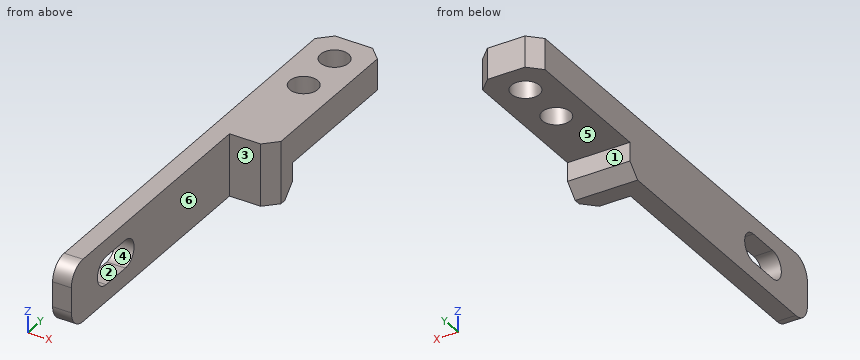
```python
from build123d import *

# Parameters (mm, degrees)
SKETCH1_W            = 10
SKETCH1_H            = 70
BOSS_EXTRUDE1_DEPTH  = 5
SKETCH2_W            = 7
SKETCH2_H            = 41
CUT_EXTRUDE1_DEPTH   = 37.742346142
SKETCH3_W            = 5
SKETCH3_H            = 24
CUT_EXTRUDE2_DEPTH   = 37.742346142
CUT_EXTRUDE3_DEPTH   = 37.742346142
FILLET1_R            = 3
M4_CLEARANCE_HOLE1_D = 4.5
CHAMFER1_SIZE        = 2


with BuildPart() as part:
    # Sketch1 → Boss-Extrude1 (new, symmetric)
    with BuildSketch(Plane.XY):
        Rectangle(SKETCH1_W, SKETCH1_H)
    extrude(amount=BOSS_EXTRUDE1_DEPTH, both=True)

    # Sketch2 → Cut-Extrude1 (cut, through all)
    with BuildSketch(Plane.XY.offset(5)):
        with Locations((1.5, -14.5)):
            Rectangle(SKETCH2_W, SKETCH2_H)
    extrude(amount=-CUT_EXTRUDE1_DEPTH, mode=Mode.SUBTRACT)

    # Sketch3 → Cut-Extrude2 (cut, through all)
    with BuildSketch(Plane(origin=(5, 0, 0), x_dir=(0, 0, -1), z_dir=(1, 0, 0))):
        with Locations((2.5, 23)):
            Rectangle(SKETCH3_W, SKETCH3_H)
    extrude(amount=-CUT_EXTRUDE2_DEPTH, mode=Mode.SUBTRACT)

    # Sketch4 → Cut-Extrude3 (cut, through all)
    with BuildSketch(Plane.ZY.offset(5)):
        with BuildLine():
            Line((2.25, -21), (2.25, -26))
            ThreePointArc((2.25, -26), (0, -28.25), (-2.25, -26))
            Line((-2.25, -26), (-2.25, -21))
            ThreePointArc((-2.25, -21), (0, -18.75), (2.25, -21))
        make_face()
    extrude(amount=-CUT_EXTRUDE3_DEPTH, mode=Mode.SUBTRACT)

    # Fillet1
    fillet1_edges = [part.edges().sort_by_distance(p)[0] for p in [
        (-3.5, -35, 5),
        (-3.5, -35, -5),
    ]]
    fillet(fillet1_edges, radius=FILLET1_R)

    # M4 Clearance Hole1 (through all)
    with Locations(Plane.XY.offset(5)):
        with Locations((0, 30), (0, 22)):
            Hole(M4_CLEARANCE_HOLE1_D / 2)

    # Chamfer1
    chamfer1_edges = [part.edges().sort_by_distance(p)[0] for p in [
        (5, 6, 0),
        (0, 11, -5),
        (-5, 35, 2.5),
        (5, 35, 2.5),
    ]]
    chamfer(chamfer1_edges, length=CHAMFER1_SIZE)


solid = part.part
```
Work out the finished part from the listing and answer in its coordinate system (mm). Face numbers are marked on the shaded views. A direction names the side the tool comes from. Give positions to 0.01 mm unless a question says otherwise; leave off trailing zeros. Write each loop counter-clockwise with the first axis right and the second up, starting at its lowest first coordinate (ties: lowest second). Pieces come first, ordered by that corner, then holes. Notation, with made-up numbers: (-15.5, -14.75) - (16.5, -14.75) arc R27 ccw to (16.5, 13.25) - close; hole circle Ø5 at (66, 9). An arc over 180 degrees is marked (long way). Use one line per item in the form item = value.
1. Each of these flat-tipped pins is pushed along its axis until it touches: pin 1 Ø3 at (x, y) = (3, 13.5) entering from -Z; pin 2 Ø6 at (y, z) = (-17.5, -3) entering from +X; pin 3 Ø5 at (x, y) = (0, 30) entering from +Z; pin 4 Ø1.5 at (x, z) = (0.5, 0) entering from -Y. Where does it stop, or does it pass through?
Filled in:
pin_1 = 0
pin_2 = -2
pin_3 = 5
pin_4 = 6
2. Consider L1, parallel to Y at x = 0, z = 1.3; L2, parallel to Z at x = -2.5, y = -25; L3, parallel to X at y = -1.5, z = 0. Determine where each line is inside the solid, lowest interval first.
Filled in:
L1 = 6 to 19.75, 24.25 to 27.75, 32.25 to 35
L2 = -5 to -2.25, 2.25 to 5
L3 = -5 to -2
3. A cutting plane is placed at D-D (x = 4). Write down the section's boundary in (y, z).
Filled in:
outline = (7, -5) - (9, -5) - (11, -3) - (11, 0) - (34, 0) - (34, 5) - (7, 5) - close
4. A cutting plane is placed at B-B (x = 0). Write down the section's boundary in (y, z).
Filled in:
outline = (6, -5) - (9, -5) - (11, -3) - (11, 0) - (19.75, 0) - (19.75, 5) - (6, 5) - close; (24.25, 0) - (27.75, 0) - (27.75, 5) - (24.25, 5) - close; (32.25, 0) - (35, 0) - (35, 5) - (32.25, 5) - close
5. A cutting plane is placed at A-A (y = 30). Write down the section's boundary in (x, z), and give its area (3 significant figures).
Filled in:
outline = (-5, 0) - (-2.25, 0) - (-2.25, 5) - (-5, 5) - close; (2.25, 0) - (5, 0) - (5, 5) - (2.25, 5) - close
area = 27.5 mm^2
6. For the marked faces 1, 2 and 3, determine the directions among +Z, -Z, +X, -X, +Y, -Y from which every point of the face is accessible in a straight line to the end or side of a thin tool.
Filled in:
face_1 = -Z, +X, -X, +Y
face_2 = +X, -X
face_3 = +Z, -Z, +X, -Y
7. A cutting plane is placed at C-C (z = 0.75). Write down the section's boundary in (x, y), and give its area (3 significant figures).
Filled in:
outline = (-5, -35) - (-2, -35) - (-2, -28.12) - (-5, -28.12) - close; (-5, -18.88) - (-2, -18.88) - (-2, 6) - (3, 6) - (5, 8) - (5, 33) - (3, 35) - (-3, 35) - (-5, 33) - close; hole circle Ø4.5 at (0, 22); hole circle Ø4.5 at (0, 30)
area = 347 mm^2
8. Determine the mould class of the marked faces 4, 5 and 6 for opening direction Z: released by +Z, released by -Z, zero draft, split by the parting line, or undercut.
Filled in:
face_4 = undercut
face_5 = released by -Z
face_6 = zero draft
